```python
from build123d import *

# Parameters (mm, degrees)
EXTRUDE_1_DEPTH     = 70
SHELL_1_T           = -5
EXTRUDE_2_DEPTH     = 5
CUT_EXTRUDE_1_DEPTH = 5
FILLET_1_R          = 10
FILLET_2_R          = 10
CUT_EXTRUDE_2_DEPTH = 5


with BuildPart() as part:
    # 草图1 → 凸台-拉伸1 (new body)
    with BuildSketch(Plane.XY):
        Polygon((0, 70), (0, -50), (595, 40), (595, 70), (570, 70), align=None)
    extrude(amount=EXTRUDE_1_DEPTH)

    # 抽壳1
    shell_1_openings = [part.faces().sort_by_distance(p)[0] for p in [
        (0, 10, 35),
        (595, 55, 35),
        (297.5, -5, 35),
    ]]
    offset(amount=SHELL_1_T, openings=shell_1_openings, kind=Kind.INTERSECTION)

    # 草图2 → 凸台-拉伸2 (add)
    with BuildSketch(Plane.XY.offset(70)):
        Polygon((465, 10), (595, 40), (396.666666667, 10), align=None)
    extrude(amount=-EXTRUDE_2_DEPTH)

    # 草图3 → 切除-拉伸1 (cut)
    with BuildSketch(Plane.XY.offset(70)):
        Polygon((0, -50), (396.666666667, 10), (0, 10), align=None)
    extrude(amount=-CUT_EXTRUDE_1_DEPTH, mode=Mode.SUBTRACT)

    # 圆角1
    fillet_1_edges = [part.edges().sort_by_distance(p)[0] for p in [
        (297.5, 70, 70),
    ]]
    fillet(fillet_1_edges, radius=FILLET_1_R)

    # 圆角2
    fillet_2_edges = [part.edges().sort_by_distance(p)[0] for p in [
        (297.5, 70, 0),
    ]]
    fillet(fillet_2_edges, radius=FILLET_2_R)

    # 草图4 → 切除-拉伸2 (cut)
    with BuildSketch(Plane(origin=(0, 70, 0), x_dir=(1, 0, 0), z_dir=(0, 1, 0))):
        with BuildLine():
            Line((160, -40), (140, -40))
            ThreePointArc((140, -40), (135, -35), (140, -30))
            Line((140, -30), (160, -30))
            ThreePointArc((160, -30), (165, -35), (160, -40))
        make_face()
        with BuildLine():
            Line((460, -30), (480, -30))
            ThreePointArc((480, -30), (485, -35), (480, -40))
            Line((480, -40), (460, -40))
            ThreePointArc((460, -40), (455, -35), (460, -30))
        make_face()
    extrude(amount=-CUT_EXTRUDE_2_DEPTH, mode=Mode.SUBTRACT)


solid = part.part
```
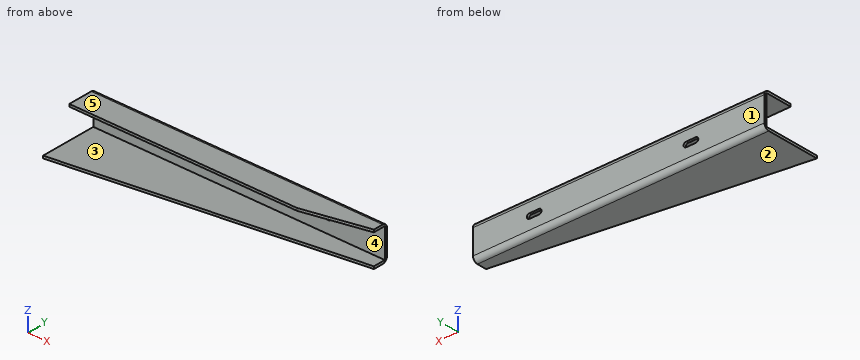
Check sheet for the modelled part. Datum: model origin and axes. Units: mm. Face numbers are marked on the shaded views. A direction names the side the tool comes from. Coordinates: 2 decimals unless noted, no trailing zeros. Write each loop counter-clockwise with the first axis right and the second up, starting at its lowest first coordinate (ties: lowest second). Pieces come first, ordered by that corner, then holes. Notation, with made-up numbers: M -40,38 L -24,38 A4 cw -24,44 Z; hole C 56.5,49.25 d9. An arc over 180 degrees is marked long. Write item = value, one per line. Start each with the question number.
1. Sectioned sample at B-B (y = 47). Record the cut outline in (x, z), then the cut area to 3 significant figures.
2. Mould release check, pull along Z, two halves, no side actions. Record for the marked faces 1, 2 and 3: pulls with the +Z half, pulls with the -Z half, needs draft (parallel to the pull), parting line crosses it, or undercut.
3. Thickness scan on probe 1 along Z at (x, y) = (250, 29); probe 2 along Z at (x, y) = (156, -9); probe 3 along Y at (x, z) = (387, 53). Record the ranges inside material, lowest first.
4. Sectioned sample at C-C (x = 171). Record the cut outline in (y, z), then the cut area to 3 significant figures.
5. Tool access check on the marked faces 4 and 5. Record the directions out of +Z, -Z, +X, -X, +Y, -Y that give a thin tool (end or side, any length) a straight path to the whole face; none if there is none.
6. Sectioned sample at A-A (z = 35). Record the cut outline in (x, y).
7. Sectioned sample at D-D (y = -14). Record the cut outline in (x, z), then the cut area to 3 significant figures.
8. Go/stop test with flat-tipped pins: pin 1 (2.5 mm diameter, centred on x = 471.5, y = 68.5, fed in from +Z); pin 2 (4 mm diameter, centred on x = 470.5, y = 67.5, fed in from -Z); pin 3 (10 mm diameter, centred on x = 463.5, z = 17.5, fed in from -Y). Record where each tip stops, or that it passes through.
The answers:
q1.outline = M 0,0 L 595,0 L 595,5 L 0,5 Z; M 0,65 L 595,65 L 595,70 L 0,70 Z
q1.area = 5,950 mm²
q2.face_1 = needs draft
q2.face_2 = pulls with the -Z half
q2.face_3 = undercut
q3.probe_1 = 0 to 5, 65 to 70
q3.probe_2 = 0 to 5
q3.probe_3 = 65 to 70
q4.outline = M -24.13,0 L 60,0 A10 ccw 70,10 L 70,60 A10 ccw 60,70 L 10,70 L 10,65 L 65,65 L 65,5 L -24.13,5 Z
q4.area = 1,030 mm²
q5.face_4 = +X, -X, -Y
q5.face_5 = +Z, +X, -X, +Y, -Y
q6.outline = M 0,65 L 135,65 L 135,70 L 0,70 Z; M 165,65 L 455,65 L 455,70 L 165,70 Z; M 485,65 L 595,65 L 595,70 L 485,70 Z
q7.outline = M 0,0 L 238,0 L 238,5 L 0,5 Z
q7.area = 1,190 mm²
q8.pin_1 = 66.89
q8.pin_2 = 1.65
q8.pin_3 = 65
